Here's how the part is built. I have some questions about the finished solid (model axes, mm). Face numbers are marked on the shaded views. A direction names the side the tool comes from. Round coordinates to 2 decimals unless told otherwise and drop trailing zeros. Order: outer loops, then holes, each group sorted by start corner. A loop starts at its lowest first (then second) coordinate and runs counter-clockwise, first axis right, second up. Notation, with made-up numbers: (25.25, 27.25) -> (52.25, 27.25) arc R15 ccw to (52.25, 40.25) -> close; hole circle Ø2 at (64.5, 55). An arc over 180 degrees is marked (long way). Use a Markdown table: item, result. Add a question column.
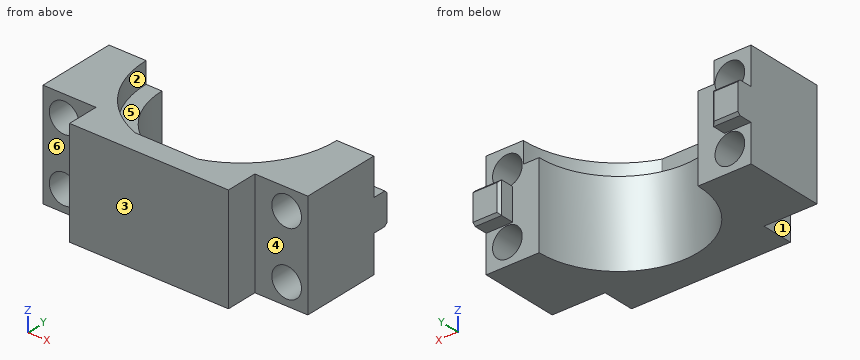
from build123d import *

# Parameters (mm, degrees)
SKETCH1_W           = 50
SKETCH1_H           = 21
BOSS_EXTRUDE1_DEPTH = 20
SKETCH2_R           = 15
CUT_EXTRUDE1_DEPTH  = 20
SKETCH3_W           = 10
SKETCH3_H           = 6
CUT_EXTRUDE2_DEPTH  = 20
SKETCH4_R           = 2.8
CUT_EXTRUDE3_DEPTH  = 20
SKETCH5_W           = 5
SKETCH5_H           = 6
BOSS_EXTRUDE2_DEPTH = 3
CHAMFER2_SIZE       = 0.5
CUT_EXTRUDE4_DEPTH  = 4


with BuildPart() as part:
    # Sketch1 → Boss-Extrude1 (new body)
    with BuildSketch(Plane.XY):
        Rectangle(SKETCH1_W, SKETCH1_H)
    extrude(amount=BOSS_EXTRUDE1_DEPTH)

    # Sketch2 → Cut-Extrude1 (cut)
    with BuildSketch(Plane.XY.offset(20)):
        with Locations((0, 10.5)):
            Circle(SKETCH2_R)
    extrude(amount=-CUT_EXTRUDE1_DEPTH, mode=Mode.SUBTRACT)

    # Sketch3 → Cut-Extrude2 (cut)
    with BuildSketch(Plane.XY.offset(20)):
        with Locations((-20, -7.5)):
            Rectangle(SKETCH3_W, SKETCH3_H)
        with Locations((20, -7.5)):
            Rectangle(SKETCH3_W, SKETCH3_H)
    extrude(amount=-CUT_EXTRUDE2_DEPTH, mode=Mode.SUBTRACT)

    # Sketch4 → Cut-Extrude3 (cut)
    with BuildSketch(Plane.XZ.offset(4.5)):
        with Locations((-21, 16)):
            Circle(SKETCH4_R)
        with Locations((-21, 4)):
            Circle(SKETCH4_R)
        with Locations((21, 16)):
            Circle(SKETCH4_R)
        with Locations((21, 4)):
            Circle(SKETCH4_R)
    extrude(amount=-CUT_EXTRUDE3_DEPTH, mode=Mode.SUBTRACT)

    # Sketch5 → Boss-Extrude2 (add)
    with BuildSketch(Plane(origin=(0, 10.5, 0), x_dir=(1, 0, 0), z_dir=(0, 1, 0))):
        with Locations((-22.5, -10)):
            Rectangle(SKETCH5_W, SKETCH5_H)
        with Locations((22.5, -10)):
            Rectangle(SKETCH5_W, SKETCH5_H)
    extrude(amount=BOSS_EXTRUDE2_DEPTH)

    # Chamfer2
    chamfer2_edges = [part.edges().sort_by_distance(p)[0] for p in [
        (-22.5, 13.5, 13),
        (-20, 13.5, 10),
        (-22.5, 13.5, 7),
        (20, 13.5, 10),
        (22.5, 13.5, 13),
        (22.5, 13.5, 7),
    ]]
    chamfer(chamfer2_edges, length=CHAMFER2_SIZE)

    # Sketch6 → Cut-Extrude4 (cut)
    with BuildSketch(Plane.XY.offset(20)):
        with BuildLine():
            Line((-5.916079783, -6.5), (5.916079783, -6.5))
            ThreePointArc((5.916079783, -6.5), (0, 28.5), (-5.916079783, -6.5))
        make_face()
    extrude(amount=-CUT_EXTRUDE4_DEPTH, mode=Mode.SUBTRACT)


solid = part.part
(1) If we mould it in two halves opening along X, with no side actions, what happens to the marked faces 1, 2 and 3? For each: pulls with the +X half, pulls with the -X half, needs draft (parallel to the pull), parting line crosses it, or undercut.
(2) I'm going to push flat-ended pins straight in: P1, Ø1.8, axis at y = -8, z = 12, coming from the +X side; P2, Ø3.5, axis at x = 21, z = 16, coming from the -Y side; P3, Ø3, axis at x = 2.5, z = 6.5, coming from the +Y side; P4, Ø1.5, axis at x = 4, z = 12.5, coming from the +Y side. Where does each tip first touch, or does it pass through?
(3) I want a section at C-C on z = 16.75. List the corners of the cut face in (x, y) for me.
(4) On a 3-axis mill with a long thin cutter (end or side, diameter ignored), from which of +Z, -Z, +X, -X, +Y, -Y can I reach the whole of each face in a straight line? I mean the marked faces 4, 5 and 6. Say none if no direction works.
(5) I want a section at A-A on x = -21. List the corners of the cut face in (y, z) for me.
(6) I want a section at B-B on y = 1.25. List the corners of the cut face in (x, z) for me, and give its area (3 significant figures).
(7) Please list where these lines run through material, in increasing order: probe 1 along Z at (x, y) = (21, 0.5); probe 2 along X at (y, z) = (3.25, 5); probe 3 along Y at (x, z) = (-18.5, 17.5). Write a range as from..to.
(8) I want a section at D-D on z = 9.75. List the corners of the cut face in (x, y) for me, and give its area (3 significant figures).
Output:
| question | item | result |
|---|---|---|
| 1 | face 1 | pulls with the -X half |
| 1 | face 2 | undercut |
| 1 | face 3 | needs draft |
| 2 | P1 | x = 15 |
| 2 | P2 | through |
| 2 | P3 | y = -3.96 |
| 2 | P4 | y = -3.73 |
| 3 | outline | (-25, -4.5) -> (-23.7, -4.5) -> (-23.7, 10.5) -> (-25, 10.5) -> close; (-18.3, -4.5) -> (-15, -4.5) -> (-15, -10.5) -> (15, -10.5) -> (15, -4.5) -> (18.3, -4.5) -> (18.3, 10.5) -> (18, 10.5) arc R18 cw to (5.92, -6.5) -> (-5.92, -6.5) arc R18 cw to (-18, 10.5) -> (-18.3, 10.5) -> close; (23.7, -4.5) -> (25, -4.5) -> (25, 10.5) -> (23.7, 10.5) -> close |
| 4 | face 4 | +Z, -Z, +X, -Y |
| 4 | face 5 | +Z, +Y |
| 4 | face 6 | +Z, -Z, -X, -Y |
| 5 | outline | (-4.5, 0) -> (10.5, 0) -> (10.5, 1.2) -> (-4.5, 1.2) -> close; (-4.5, 6.8) -> (10.5, 6.8) -> (10.5, 7) -> (13, 7) -> (13.5, 7.5) -> (13.5, 12.5) -> (13, 13) -> (10.5, 13) -> (10.5, 13.2) -> (-4.5, 13.2) -> close; (-4.5, 18.8) -> (10.5, 18.8) -> (10.5, 20) -> (-4.5, 20) -> close |
| 6 | outline | (-25, 0) -> (-11.81, 0) -> (-11.81, 16) -> (-15.44, 16) -> (-15.44, 20) -> (-25, 20) -> close; (11.81, 0) -> (25, 0) -> (25, 20) -> (15.44, 20) -> (15.44, 16) -> (11.81, 16) -> close; hole circle Ø5.6 at (-21, 4); hole circle Ø5.6 at (-21, 16); hole circle Ø5.6 at (21, 4); hole circle Ø5.6 at (21, 16) |
| 6 | area | 400 mm² |
| 7 | probe 1 | 0..1.2, 6.8..13.2, 18.8..20 |
| 7 | probe 2 | -25..-23.62, -18.38..-13.13, 13.13..18.38, 23.62..25 |
| 7 | probe 3 | -4.5..10.5 |
| 8 | outline | (-25, -4.5) -> (-15, -4.5) -> (-15, -10.5) -> (15, -10.5) -> (15, -4.5) -> (25, -4.5) -> (25, 13.5) -> (20.5, 13.5) -> (20, 13) -> (20, 10.5) -> (15, 10.5) arc R15 cw to (-15, 10.5) -> (-20, 10.5) -> (-20, 13) -> (-20.5, 13.5) -> (-25, 13.5) -> close |
| 8 | area | 606 mm² |
